Verification items for the finished model (mm, model axes). Give positions to 0.01 mm unless a question says otherwise; leave off trailing zeros. Write each loop counter-clockwise with the first axis right and the second up, starting at its lowest first coordinate (ties: lowest second). Pieces come first, ordered by that corner, then holes. Notation, with made-up numbers: (56, 35) -> (92, 35) arc R16 cw to (92, 54) -> close; hole circle Ø4 at (-30, 5.5). An arc over 180 degrees is marked (long way). Answer as CSV lines item,"result".
```python
from build123d import *

# Parameters (mm, degrees)
SKETCH1_R           = 10
SKETCH1_R_2         = 17.5
BOSS_EXTRUDE1_DEPTH = 3


with BuildPart() as part:
    # Sketch1 → Boss-Extrude1 (new body)
    with BuildSketch(Plane.XY):
        with BuildLine():
            Line((0, 587), (0, 45))
            ThreePointArc((0, 45), (-13.180194847, 13.180194847), (-45, 0))
            Line((-45, 0), (-742.749907476, 0))
            ThreePointArc((-742.749907476, 0), (-793.219621271, 6.644463874), (-840.249907476, 26.125046262))
            Line((-840.249907476, 26.125046262), (-1041.5, 142.316841355))
            ThreePointArc((-1041.5, 142.316841355), (-1112.874953738, 213.691795093), (-1139, 311.191795093))
            Line((-1139, 311.191795093), (-1139, 587))
            Line((-1139, 587), (0, 587))
        make_face()
        with Locations((-650, 300)):
            Circle(SKETCH1_R, mode=Mode.SUBTRACT)
        with Locations((-150, 300)):
            Circle(SKETCH1_R, mode=Mode.SUBTRACT)
        with Locations((-940, 257)):
            Circle(SKETCH1_R_2, mode=Mode.SUBTRACT)
    extrude(amount=BOSS_EXTRUDE1_DEPTH)


solid = part.part
```
1) Depth check by flat-ended pin: pin 1 (2 mm diameter, centred on x = -442, y = 336.5, fed in from -Z); pin 2 (1.5 mm diameter, centred on x = -954, z = 1.5, fed in from -Y); pin 3 (1.5 mm diameter, centred on y = 165.5, z = 0.5, fed in from -X). Enter the tip coordinate at first touch or a pass-through.
Reported:
pin 1,"z = 0"
pin 2,"y = 91.37"
pin 3,"x = -1074.45"
2) Section check A-A (z = 2.25). Record the boundary of the cut face in (x, y), and give its area (3 significant figures).
Reported:
outline,"(-1139, 311.19) arc R195 ccw to (-1041.5, 142.32) -> (-840.25, 26.13) arc R195 ccw to (-742.75, 0) -> (-45, 0) arc R45 ccw to (0, 45) -> (0, 587) -> (-1139, 587) -> close; hole circle Ø35 at (-940, 257); hole circle Ø20 at (-650, 300); hole circle Ø20 at (-150, 300)"
area,"630,000 mm²"
3) Section check B-B (x = -940). Record the boundary of the cut face in (y, z).
Reported:
outline,"(83.72, 0) -> (239.5, 0) -> (239.5, 3) -> (83.72, 3) -> close; (274.5, 0) -> (587, 0) -> (587, 3) -> (274.5, 3) -> close"
4) Scan lines: line 1 along Y through (x, z) = (-650, 0.95); line 2 along Y through (x, z) = (-940, 0.8); line 3 along Y through (x, z) = (-879, 2.75). Record each from-to range of solid material in increasing order.
Reported:
line 1,"0 to 290, 310 to 587"
line 2,"83.72 to 239.5, 274.5 to 587"
line 3,"48.5 to 587"
5) Draft check along Y on faces 1 (the flat face through (-562, 298, 0)), 2 (the cylindrical face through (-640.763, 296.17, 1.479)), 3 (the flat face through (-939.47, 83.41, 1.48)). Enter one of: +Y half, -Y half, draft (parallel to the pull), parting line (faces both ways), or undercut.
Reported:
face 1,"draft"
face 2,"undercut"
face 3,"-Y half"
6) Section check C-C (y = 257). Record the boundary of the cut face in (x, z).
Reported:
outline,"(-1131.32, 0) -> (-957.5, 0) -> (-957.5, 3) -> (-1131.32, 3) -> close; (-922.5, 0) -> (0, 0) -> (0, 3) -> (-922.5, 3) -> close"
